Geometry: final body of the model. Coordinates: model frame, mm. A direction names the side the tool comes from. Give positions to 0.01 mm unless a question says otherwise; leave off trailing zeros. Order: outer loops, then holes, each group sorted by start corner. A loop starts at its lowest first (then second) coordinate and runs counter-clockwise, first axis right, second up. Notation, with made-up numbers: (25, 78) - (77, 78) arc R22 cw to (77, 90) - close; hole circle Ø9 at (73, 14). An arc over 180 degrees is marked (long way). One line per item, written item: value.
```python
from build123d import *

# Parameters (mm, degrees)
SKETCH_1_W                = 210
SKETCH_1_H                = 130
EXTRUDE_1_DEPTH           = 20
SKETCH_2_W                = 210
SKETCH_2_H                = 50
EXTRUDE_2_DEPTH           = 252
SKETCH_3_R                = 26
CUT_EXTRUDE_1_DEPTH       = 15
SKETCH_4_R                = 17.5
CUT_EXTRUDE_2_DEPTH       = 302.054812285
SKETCH_5_W                = 160
SKETCH_5_H                = 41
CUT_EXTRUDE_3_DEPTH       = 150
HOLE_WIZARD_M8_1_D        = 6.8
HOLE_WIZARD_M8_1_DEPTH    = 19.75
HOLE_WIZARD_M8_1_TIP      = 2.042926105
HOLE_WIZARD_10_5_10_5_1_D = 10.5
SKETCH_10_W               = 150
SKETCH_10_H               = 40
CUT_EXTRUDE_4_DEPTH       = 281.631430884
HOLE_WIZARD_12_5_12_5_1_D = 12.5
CHAMFER_1_SIZE            = 5
FILLET_1_R                = 5


with BuildPart() as part:
    # 草图1 → 凸台-拉伸1 (new body)
    with BuildSketch(Plane(origin=(0, 0, 0), x_dir=(0, 0, -1), z_dir=(1, 0, 0))):
        Rectangle(SKETCH_1_W, SKETCH_1_H)
    extrude(amount=EXTRUDE_1_DEPTH)

    # 草图2 → 凸台-拉伸2 (add)
    with BuildSketch(Plane(origin=(20, 0, 0), x_dir=(0, 0, -1), z_dir=(1, 0, 0))):
        Rectangle(SKETCH_2_W, SKETCH_2_H)
    extrude(amount=EXTRUDE_2_DEPTH)

    # 草图3 → 切除-拉伸1 (cut)
    with BuildSketch(Plane(origin=(0, 25, 0), x_dir=(1, 0, 0), z_dir=(0, 1, 0))):
        with Locations(Location((74, 0, 0), (0, 0, 270))):
            Circle(SKETCH_3_R)
    extrude(amount=-CUT_EXTRUDE_1_DEPTH, mode=Mode.SUBTRACT)

    # 草图4 → 切除-拉伸2 (cut, through all)
    with BuildSketch(Plane(origin=(0, 10, 0), x_dir=(1, 0, 0), z_dir=(0, 1, 0))):
        with Locations(Location((74, 0, 0), (0, 0, 270))):
            Circle(SKETCH_4_R)
    extrude(amount=-CUT_EXTRUDE_2_DEPTH, mode=Mode.SUBTRACT)

    # 草图5 → 切除-拉伸3 (cut)
    with BuildSketch(Plane(origin=(272, 0, 0), x_dir=(0, 0, -1), z_dir=(1, 0, 0))):
        with Locations((0, 4.5)):
            Rectangle(SKETCH_5_W, SKETCH_5_H)
    extrude(amount=-CUT_EXTRUDE_3_DEPTH, mode=Mode.SUBTRACT)

    # M8 螺纹孔1
    with Locations(Plane(origin=(272, 0, 0), x_dir=(0, 0, -1), z_dir=(1, 0, 0))):
        with Locations((-87.5, 0), (87.5, 0)):
            Hole(HOLE_WIZARD_M8_1_D / 2, depth=HOLE_WIZARD_M8_1_DEPTH)
            with Locations((0, 0, -(HOLE_WIZARD_M8_1_DEPTH + HOLE_WIZARD_M8_1_TIP / 2))):  # 118° drill point
                Cone(0, HOLE_WIZARD_M8_1_D / 2, HOLE_WIZARD_M8_1_TIP, mode=Mode.SUBTRACT)

    # Ø10.5 (10.5) 直径孔1 (through all)
    with Locations(Plane(origin=(0, -25, 0), x_dir=(-1, 0, 0), z_dir=(0, -1, 0))):
        with Locations((-134, 30), (-134, -30)):
            Hole(HOLE_WIZARD_10_5_10_5_1_D / 2)

    # 草图10 → 切除-拉伸4 (cut, through all)
    with BuildSketch(Plane(origin=(20, 0, 0), x_dir=(0, 0, -1), z_dir=(1, 0, 0))):
        with Locations((0, -45)):
            Rectangle(SKETCH_10_W, SKETCH_10_H)
    extrude(amount=-CUT_EXTRUDE_4_DEPTH, mode=Mode.SUBTRACT)

    # Ø12.5 (12.5) 直径孔1 (through all)
    with Locations(Plane(origin=(20, 0, 0), x_dir=(0, 0, -1), z_dir=(1, 0, 0))):
        with Locations((-90, 45), (0, 45), (90, 45), (-90, -45), (90, -45)):
            Hole(HOLE_WIZARD_12_5_12_5_1_D / 2)

    # 倒角1
    chamfer_1_edges = [part.edges().sort_by_distance(p)[0] for p in [
        (10, -65, -105),
        (10, -65, 105),
        (10, -65, 75),
        (10, 65, 105),
        (10, -65, -75),
        (10, 65, -105),
    ]]
    chamfer(chamfer_1_edges, length=CHAMFER_1_SIZE)

    # 圆角1
    fillet_1_edges = [part.edges().sort_by_distance(p)[0] for p in [
        (122, 4.5, 80),
        (122, 4.5, -80),
    ]]
    fillet(fillet_1_edges, radius=FILLET_1_R)


solid = part.part
```
1) Mould query, pull axis Z, two halves, no side actions, for faces 5 (the face through (69, 10, 17)), 6 (the face through (104, -1, 105)), 7 (the face through (10, -65, -90)). Classes: released by +Z, released by -Z, zero draft, split by the parting line, or undercut.
Answers below:
face 5: undercut
face 6: released by +Z
face 7: zero draft
2) Section D-D, the plane x = 212. Return loops of the section in (y, z), then the cut area to 3 significant figures.
Answers below:
outline: (-25, -105) - (25, -105) - (25, -80) - (-16, -80) - (-16, 80) - (25, 80) - (25, 105) - (-25, 105) - close
area: 3,940 mm^2
3) Section A-A, the plane z = 30. Return loops of the section in (x, y), then the cut area to 3 significant figures.
Answers below:
outline: (0, -25) - (128.75, -25) - (128.75, -16) - (122, -16) - (122, 25) - (20, 25) - (20, 65) - (0, 65) - close; (139.25, -25) - (272, -25) - (272, -16) - (139.25, -16) - close
area: 8,160 mm^2
4) Section B-B, the plane y = -45. Return loops of the section in (x, z).
Answers below:
outline: (0, -105) - (20, -105) - (20, -96.25) - (0, -96.25) - close; (0, -83.75) - (20, -83.75) - (20, -75) - (0, -75) - close; (0, 75) - (20, 75) - (20, 83.75) - (0, 83.75) - close; (0, 96.25) - (20, 96.25) - (20, 105) - (0, 105) - close
5) Material intervals for line 1 along Y through (x, z) = (5, -90); line 2 along Z through (x, y) = (134, -19.5); line 3 along Z through (x, y) = (152, -4), sorted ascending.
Answers below:
line 1: -65 to -51.25, -38.75 to 38.75, 51.25 to 65
line 2: -105 to -35.25, -24.75 to 24.75, 35.25 to 105
line 3: -105 to -80, 80 to 105
6) Section C-C, the plane z = 0. Return loops of the section in (x, y).
Answers below:
outline: (0, -25) - (56.5, -25) - (56.5, 10) - (48, 10) - (48, 25) - (20, 25) - (20, 38.75) - (0, 38.75) - close; (0, 51.25) - (20, 51.25) - (20, 65) - (0, 65) - close; (91.5, -25) - (272, -25) - (272, -16) - (122, -16) - (122, 25) - (100, 25) - (100, 10) - (91.5, 10) - close
7) First-contact query: pin 1 (10 mm diameter, centred on y = -45, z = 90, fed in from -X); pin 2 (1 mm diameter, centred on x = 103, z = -69, fed in from -Y); pin 3 (24 mm diameter, centred on y = -45, z = -83.5, fed in from +X); pin 4 (5 mm diameter, centred on y = 14.5, z = 17.5, fed in from +X). Flat tips, straight axial feed; report the tip coordinate or a pass-through.
Answers below:
pin 1: through
pin 2: y = -25
pin 3: x = 20
pin 4: x = 122
8) Set-up query: faces 1 (the face through (261.987, -2.069, -90.198)), 2 (the face through (20, -45, 97)), 3 (the face through (116, 25, 1)), 4 (the face through (198, -16, 1)). Return all of +Z, -Z, +X, -X, +Y, -Y with unobstructed straight access to the full face (end or side cutting, diameter ignored); none if empty.
Answers below:
face 1: +X
face 2: +Z, -Z, +X, -Y
face 3: +Z, -Z, +X, +Y
face 4: +X, +Y
